Can you work these out from the model? Positions are in its coordinate system, mm. A direction names the side the tool comes from. Round coordinates to 2 decimals unless told otherwise and drop trailing zeros. Write each loop counter-clockwise with the first axis right and the second up, starting at its lowest first coordinate (ties: lowest second). Pieces come first, ordered by that corner, then holes.
Q1. I'm going to push flat-ended pins straight in: pin 1 Ø2 at (x, y) = (115.5, -3.5) entering from +Z; pin 2 Ø1.5 at (x, y) = (215, 1) entering from +Z; pin 3 Ø1 at (x, z) = (144, -4) entering from -Y. Where does each tip first touch, or does it pass through?
Q2. For faces 1 (the flat face through (232.5, -4, 4)), 2 (the cylindrical face through (1, 0, -5)), 3 (the flat face through (199.5, -6, -2)), which set-ups out of +Z, -Z, +X, -X, +Y, -Y let a thin tool reach every point of the face, with its end or its side?
Q3. Please list where these lines run through material, in increasing order: line 1 along X through (y, z) = (0.5, -5.75); line 2 along X through (y, z) = (1, -7); line 3 along Y through (x, z) = (235, -0.5).
Q4. We'd pull the mould along X, two halves only. Please class faces 4 (the flat face through (236.5, -4, -4)), 5 (the cylindrical face through (105.83, 7.81, -1.73)), 6 (the flat face through (0, 0, 0)), 7 (the flat face through (228.5, -4, -4)): +X half, -X half, draft (parallel to the pull), parting line (faces both ways), or undercut.
Q5. If we section it at A-A (x = 100.5): Please give me the cut outline in (y, z), plus the area to 3 significant figures.
from build123d import *

# Parameters (mm, degrees)
SKETCH2_OUTSIDE_W   = 68.204
SKETCH2_OUTSIDE_H   = 68.204
SKETCH2_OUTSIDE_W_2 = 22.970489672
SKETCH2_OUTSIDE_H_2 = 14
CUT_EXTRUDE1_DEPTH  = 5
CHAMFER1_SIZE       = 0.5


with BuildPart() as part:
    # Sketch1 → Revolve1 (revolve)
    with BuildSketch(Plane.XY, mode=Mode.PRIVATE) as revolve1_sk:
        Polygon((0, 0), (0, 5), (1.85, 5), (1.85, 4.8), (3, 4.8), (3, 5), (9.5, 5), (9.5, 8), (199.5, 8), (199.5, 6), (228.5, 6), (228.5, 5), (232.5, 5), (232.5, 6), (236.5, 6), (236.5, 5), (250, 5), (250, 0), align=None)
    revolve(revolve1_sk.sketch.rotate(Axis((0, 0, 0), (1, 0, 0)), 90), axis=Axis((0, 0, 0), (1, 0, 0)))

    # Sketch2 outside → Cut-Extrude1 (cut)
    with BuildSketch(Plane.ZY.offset(-9.5)):
        Rectangle(SKETCH2_OUTSIDE_W, SKETCH2_OUTSIDE_H)
        Rectangle(SKETCH2_OUTSIDE_W_2, SKETCH2_OUTSIDE_H_2, mode=Mode.SUBTRACT)
    extrude(amount=-CUT_EXTRUDE1_DEPTH, mode=Mode.SUBTRACT)

    # Chamfer1
    chamfer1_edges = [part.edges().sort_by_distance(p)[0] for p in [
        (250, 0, -5),
        (0, 0, -5),
    ]]
    chamfer(chamfer1_edges, length=CHAMFER1_SIZE)


solid = part.part
A:
1. pin 1: stops at z = 7.6
1. pin 2: stops at z = 5.99
1. pin 3: stops at y = -7.19
2. face 1: none
2. face 2: -X
2. face 3: +X
3. line 1: x = 9.5 to 228.5, 232.5 to 236.5
3. line 2: x = 9.5 to 199.5
3. line 3: y = -5.98 to 5.98
4. face 4: +X half
4. face 5: draft
4. face 6: -X half
4. face 7: undercut
5. outline: circle Ø16 at (0, 0)
5. area: 201 mm2
